Geometry check sheet. Reference: the model listing, model coordinates, mm. A direction names the side the tool comes from. Round coordinates to 2 decimals unless told otherwise and drop trailing zeros. Order: outer loops, then holes, each group sorted by start corner. A loop starts at its lowest first (then second) coordinate and runs counter-clockwise, first axis right, second up.
(1) Set-up check for faces 1 (the face through (29, -8, 21)), 2 (the face through (-30, 0, 18)), 3 (the face through (28.7, -13.16, 10.83)), 4 (the face through (27.6, 12.1, 9.5)): record each of +Z, -Z, +X, -X, +Y, -Y from which the full face is reachable in a straight line by a thin tool's end or side.
(2) Cross-section at D-D on z = 17. Enter the section's corners in (x, y).
(3) Gauge pin test, flat ends, axial feed: P1, Ø8, axis at y = -9, z = 6.5, coming from the -X side; P2, Ø4, axis at x = -4.5, y = -3.5, coming from the +Z side; P3, Ø0.8, axis at y = 13.5, z = 21, coming from the +X side. Record the tip position at first contact, or that the pin passes through.
(4) Thickness scan on L1, parallel to X at y = -2.25, z = 20; L2, parallel to X at y = -8.5, z = 20.25; L3, parallel to Y at x = 25.5, z = 17.25. Record the ranges inside material, lowest first.
(5) Draft check along Y on faces 5 (the face through (-28.66, -13.2, 10.83)), 6 (the face through (-28, 12, 19.3)), 7 (the face through (28.66, 13.2, 10.83)). Enter one of: pulls with the +Y half, pulls with the -Y half, needs draft (parallel to the pull), parting line crosses it, or undercut.
(6) Cross-section at C-C on y = 4. Enter the section's corners in (x, z), and give its area (3 significant figures).
(7) Cross-section at B-B on x = -2. Enter the section's corners in (y, z).
(8) Cross-section at A-A on z = 8.5. Enter the section's corners in (x, y), and give its area (3 significant figures).
from build123d import *

# Parameters (mm, degrees)
EXTRUDE_1_DEPTH       = 23
EXTRUDE_START         = 1
EXTRUDE_2_DEPTH       = 1
CUT_EXTRUDE_1_DEPTH   = 20
SKETCH_5_W            = 3.764983414
SKETCH_5_H            = 10.4
CUT_EXTRUDE_3_DEPTH   = 10
CUT_EXTRUDE_START     = 6.8
CUT_EXTRUDE_4_DEPTH   = 3.4
MIRROR_START          = 6.8
MIRROR_2_COPY_1_DEPTH = 3.4
FILLET_2_R            = 0.3
EXTRUDE_3_DEPTH       = 19.3
EXTRUDE_START_2       = -24
EXTRUDE_4_DEPTH       = 24
CUT_EXTRUDE_START_2   = -10
CUT_EXTRUDE_5_DEPTH   = 10
EXTRUDE_START_3       = -2.2
EXTRUDE_5_DEPTH       = 2.2
CUT_EXTRUDE_6_DEPTH   = 5
CUT_EXTRUDE_7_DEPTH   = 3


with BuildPart() as part:
    # 草图1 → 凸台-拉伸1 (new body)
    with BuildSketch(Plane.XY):
        with BuildLine():
            Line((-26.7, 14), (26.7, 14))
            ThreePointArc((26.7, 14), (28.679898987, 13.179898987), (29.5, 11.2))
            Line((29.5, 11.2), (29.5, -11.2))
            ThreePointArc((29.5, -11.2), (28.679898987, -13.179898987), (26.7, -14))
            Line((26.7, -14), (-26.7, -14))
            ThreePointArc((-26.7, -14), (-28.679898987, -13.179898987), (-29.5, -11.2))
            Line((-29.5, -11.2), (-29.5, 11.2))
            ThreePointArc((-29.5, 11.2), (-28.679898987, 13.179898987), (-26.7, 14))
        make_face()
        with BuildLine():
            Line((-26.7, 13), (26.7, 13))
            ThreePointArc((26.7, 13), (27.972792206, 12.472792206), (28.5, 11.2))
            Line((28.5, 11.2), (28.5, -11.2))
            ThreePointArc((28.5, -11.2), (27.972792206, -12.472792206), (26.7, -13))
            Line((26.7, -13), (-26.7, -13))
            ThreePointArc((-26.7, -13), (-27.972792206, -12.472792206), (-28.5, -11.2))
            Line((-28.5, -11.2), (-28.5, 11.2))
            ThreePointArc((-28.5, 11.2), (-27.972792206, 12.472792206), (-26.7, 13))
        make_face(mode=Mode.SUBTRACT)
    extrude(amount=EXTRUDE_1_DEPTH)

    # 草图2 → 凸台-拉伸2 (add)
    with BuildSketch(Plane(origin=(0, 0, 0), x_dir=(-1, 0, 0), z_dir=(0, 0, -1)).offset(EXTRUDE_START)):
        with BuildLine():
            Line((26.7, 14), (-26.7, 14))
            ThreePointArc((-26.7, 14), (-28.679898987, 13.179898987), (-29.5, 11.2))
            Line((-29.5, 11.2), (-29.5, -11.2))
            ThreePointArc((-29.5, -11.2), (-28.679898987, -13.179898987), (-26.7, -14))
            Line((-26.7, -14), (26.7, -14))
            ThreePointArc((26.7, -14), (28.679898987, -13.179898987), (29.5, -11.2))
            Line((29.5, -11.2), (29.5, 11.2))
            ThreePointArc((29.5, 11.2), (28.679898987, 13.179898987), (26.7, 14))
        make_face()
    extrude(amount=-EXTRUDE_2_DEPTH)

    # 草图3 → 切除-拉伸1 (cut)
    with BuildSketch(Plane.ZY.offset(29.5)):
        with BuildLine():
            Line((14, 8), (25.240812318, 8))
            Line((25.240812318, 8), (25.240812318, 0))
            Line((25.240812318, 0), (14, 0))
            ThreePointArc((14, 0), (10, 4), (14, 8))
        make_face()
    extrude(amount=-CUT_EXTRUDE_1_DEPTH, mode=Mode.SUBTRACT)

    # 草图5 → 切除-拉伸3 (cut)
    with BuildSketch(Plane.ZY.offset(29.5)):
        with Locations((23.882491707, 4)):
            Rectangle(SKETCH_5_W, SKETCH_5_H)
    extrude(amount=-CUT_EXTRUDE_3_DEPTH, mode=Mode.SUBTRACT)

    # 草图6 → 切除-拉伸4 (cut)
    with BuildSketch(Plane(origin=(0, 0, 0), x_dir=(1, 0, 0), z_dir=(0, 1, 0)).offset(CUT_EXTRUDE_START)):
        Polygon((-28.5, -21.9), (-29.2, -21.9), (-29.2, -21.55), (-28.781434231, -20.4), (-28.5, -20.4), align=None)
    cut_extrude_4 = extrude(amount=CUT_EXTRUDE_4_DEPTH, mode=Mode.SUBTRACT)

    # 镜向1: 切除-拉伸4 across plane
    add(cut_extrude_4.mirror(Plane.ZX), mode=Mode.SUBTRACT)

    # 镜向2: 切除-拉伸4 across plane
    add(cut_extrude_4.mirror(Plane(origin=(0, 0, 0), x_dir=(0, 0, 1), z_dir=(1, 0, 0))), mode=Mode.SUBTRACT)

    # 镜向2 copy 1 sketch → 镜向2 copy 1 (cut)
    with BuildSketch(Plane(origin=(0, 0, 0), x_dir=(-1, 0, 0), z_dir=(0, -1, 0)).offset(MIRROR_START)):
        Polygon((-28.5, -21.9), (-29.2, -21.9), (-29.2, -21.55), (-28.781434231, -20.4), (-28.5, -20.4), align=None)
    extrude(amount=MIRROR_2_COPY_1_DEPTH, mode=Mode.SUBTRACT)

    # 圆角2
    fillet_2_edges = [part.edges().sort_by_distance(p)[0] for p in [
        (-29, 0, 22),
        (-29, 8, 22),
    ]]
    fillet(fillet_2_edges, radius=FILLET_2_R)

    # 草图9 → 凸台-拉伸3 (add)
    with BuildSketch(Plane.XY):
        with BuildLine():
            Line((-28.5, 11.2), (-26.7, 13))
            ThreePointArc((-26.7, 13), (-27.972792206, 12.472792206), (-28.5, 11.2))
        make_face()
        with BuildLine():
            Line((28.5, 11.2), (26.7, 13))
            ThreePointArc((26.7, 13), (27.972792206, 12.472792206), (28.5, 11.2))
        make_face()
        with BuildLine():
            Line((28.5, -11.2), (26.7, -13))
            ThreePointArc((26.7, -13), (27.972792206, -12.472792206), (28.5, -11.2))
        make_face()
        with BuildLine():
            Line((-28.5, -11.2), (-26.7, -13))
            ThreePointArc((-26.7, -13), (-27.972792206, -12.472792206), (-28.5, -11.2))
        make_face()
    extrude(amount=EXTRUDE_3_DEPTH)

    # 草图11 → 凸台-拉伸4 (add)
    with BuildSketch(Plane.XY.offset(23).offset(EXTRUDE_START_2)):
        with BuildLine():
            Line((-30.7, -3.068055681), (-30.7, 11.5))
            ThreePointArc((-30.7, 11.5), (-29.967766953, 13.267766953), (-28.2, 14))
            Line((-28.2, 14), (-26.7, 14))
            ThreePointArc((-26.7, 14), (-28.679898987, 13.179898987), (-29.5, 11.2))
            Line((-29.5, 11.2), (-29.5, -7.286930049))
            ThreePointArc((-29.5, -7.286930049), (-29.639971651, -6.238034848), (-30.050090571, -5.262547444))
            Line((-30.050090571, -5.262547444), (-30.149909429, -5.092438287))
            ThreePointArc((-30.149909429, -5.092438287), (-30.560028349, -4.116950882), (-30.7, -3.068055681))
        make_face()
    extrude(amount=EXTRUDE_4_DEPTH)

    # 草图12 → 切除-拉伸5 (cut)
    with BuildSketch(Plane(origin=(-29.5, 0, 0), x_dir=(0, 0, -1), z_dir=(1, 0, 0)).offset(CUT_EXTRUDE_START_2)):
        with BuildLine():
            Line((-23, 9.2), (-23, -1.2))
            Line((-23, -1.2), (-22, -1.2))
            Line((-22, -1.2), (-22, -0.3))
            ThreePointArc((-22, -0.3), (-21.912132034, -0.087867966), (-21.7, 0))
            Line((-21.7, 0), (-14, 0))
            ThreePointArc((-14, 0), (-10, 4), (-14, 8))
            Line((-14, 8), (-21.7, 8))
            ThreePointArc((-21.7, 8), (-21.912132034, 8.087867966), (-22, 8.3))
            Line((-22, 8.3), (-22, 9.2))
            Line((-22, 9.2), (-23, 9.2))
        make_face()
    extrude(amount=CUT_EXTRUDE_5_DEPTH, mode=Mode.SUBTRACT)

    # 草图13 → 凸台-拉伸5 (add)
    with BuildSketch(Plane.XZ.offset(-8).offset(EXTRUDE_START_3)):
        Polygon((-28.5, 20.4), (-28.5, 21.9), (-29.2, 21.9), (-29.2, 21.55), (-28.781434231, 20.4), align=None)
    extrude(amount=EXTRUDE_5_DEPTH)

    # 草图14 → 切除-拉伸6 (cut)
    with BuildSketch(Plane.ZY.offset(29.2)):
        with BuildLine():
            Line((21.7, 8), (22.114153774, 8))
            Line((22.114153774, 8), (22, 8.3))
            ThreePointArc((22, 8.3), (21.912132034, 8.087867966), (21.7, 8))
        make_face()
    extrude(amount=-CUT_EXTRUDE_6_DEPTH, mode=Mode.SUBTRACT)

    # 草图10 → 切除-拉伸7 (cut, symmetric)
    with BuildSketch(Plane.ZY):
        Polygon((21.9, -13.7), (21.9, -13), (20.4, -13), (20.4, -13.281434231), (21.55, -13.7), align=None)
    cut_extrude_7 = extrude(amount=CUT_EXTRUDE_7_DEPTH, both=True, mode=Mode.SUBTRACT)

    # 镜向3: 切除-拉伸7 across plane
    add(cut_extrude_7.mirror(Plane.ZX), mode=Mode.SUBTRACT)


solid = part.part
Found:
1. face 1: none
1. face 2: +Z, -X
1. face 3: +Z, -Z, +X, -Y
1. face 4: +Z
2. outline: (-30.7, -3.07) arc R4 ccw to (-30.15, -5.09) - (-30.05, -5.26) arc R4 cw to (-29.5, -7.29) - (-29.5, -11.2) arc R2.8 ccw to (-26.7, -14) - (26.7, -14) arc R2.8 ccw to (29.5, -11.2) - (29.5, 11.2) arc R2.8 ccw to (26.7, 14) - (-28.2, 14) arc R2.5 ccw to (-30.7, 11.5) - (-30.7, 8) - (-28.5, 8) - (-28.5, 11.2) - (-26.7, 13) - (26.7, 13) - (28.5, 11.2) - (28.5, -11.2) - (26.7, -13) - (-26.7, -13) - (-28.5, -11.2) - (-28.5, 0) - (-30.7, 0) - close
3. P1: stops at x = -30.2
3. P2: stops at z = 0
3. P3: stops at x = 28.76
4. L1: x = -30.7 to -28.5, 28.5 to 29.5
4. L2: x = -29.5 to -28.5, 28.5 to 29.5
4. L3: y = -14 to -13, 13 to 14
5. face 5: pulls with the -Y half
5. face 6: undercut
5. face 7: pulls with the +Y half
6. outline: (-30.7, -1) - (29.5, -1) - (29.5, 23) - (28.5, 23) - (28.5, 0) - (-28.5, 0) - (-28.5, 10) - (-30.7, 10) - close
6. area: 105 mm2
7. outline: (-14, -1) - (14, -1) - (14, 23) - (13, 23) - (13, 21.9) - (13.7, 21.9) - (13.7, 21.55) - (13.28, 20.4) - (13, 20.4) - (13, 0) - (-13, 0) - (-13, 20.4) - (-13.28, 20.4) - (-13.7, 21.55) - (-13.7, 21.9) - (-13, 21.9) - (-13, 23) - (-14, 23) - close
8. outline: (-30.7, -3.07) arc R4 ccw to (-30.15, -5.09) - (-30.05, -5.26) arc R4 cw to (-29.5, -7.29) - (-29.5, -11.2) arc R2.8 ccw to (-26.7, -14) - (26.7, -14) arc R2.8 ccw to (29.5, -11.2) - (29.5, 11.2) arc R2.8 ccw to (26.7, 14) - (-28.2, 14) arc R2.5 ccw to (-30.7, 11.5) - close; hole (-28.5, -11.2) - (-26.7, -13) - (26.7, -13) - (28.5, -11.2) - (28.5, 11.2) - (26.7, 13) - (-26.7, 13) - (-28.5, 11.2) - close
8. area: 193 mm2
